Work out the finished part from the listing and answer in its coordinate system (mm). Face numbers are marked on the shaded views. A direction names the side the tool comes from. Round coordinates to 2 decimals unless told otherwise and drop trailing zeros. Loops run counter-clockwise (first coordinate to the right, second up) from the corner with the lowest first, then second, coordinate; pieces in that order, holes last. Notation, with made-up numbers: (48.25, -28.5) - (71.25, -28.5) arc R30 ccw to (71.25, 7.5) - close; hole circle Ø3 at (37.5, 49.5). An arc over 180 degrees is marked (long way). Use CSV: the item, a comma, the result in double quotes. Start each with the question number.
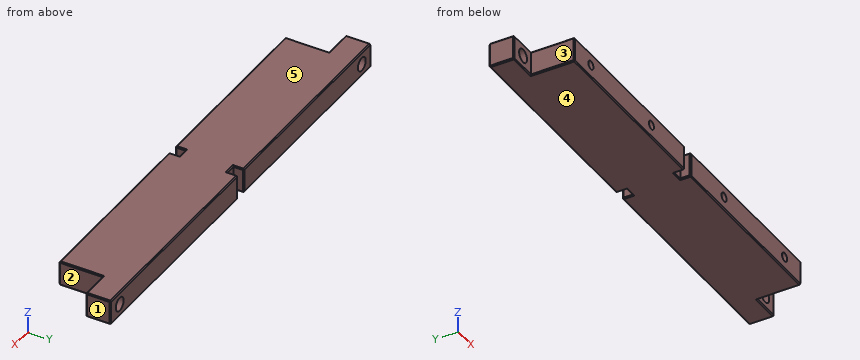
from build123d import *

# Parameters (mm, degrees)
SKETCH_1_W              = 187
SKETCH_1_H              = 33
EXTRUDE_1_DEPTH         = 12
HOLE_WIZARD_M5_1_D      = 4.2
HOLE_WIZARD_M5_1_DEPTH  = 12.4
HOLE_WIZARD_M5_1_TIP    = 1.2618073
SKETCH_8_W              = 5
SKETCH_8_H              = 12
CUT_EXTRUDE_2_DEPTH     = 5
SKETCH_11_W             = 5
SKETCH_11_H             = 5
CUT_EXTRUDE_3_DEPTH     = 96.700052247
SKETCH_12_W             = 14
SKETCH_12_H             = 12
EXTRUDE_2_DEPTH         = 12
HOLE_WIZARD_6_5_6_5_1_D = 6.5
CHAMFER_1_SIZE          = 0.5


with BuildPart() as part:
    # 草图1 → 凸台-拉伸1 (new body)
    with BuildSketch(Plane.XY):
        Rectangle(SKETCH_1_W, SKETCH_1_H)
    extrude(amount=EXTRUDE_1_DEPTH)

    # M5 螺纹孔1
    with Locations(Plane(origin=(0, -16.5, 0), x_dir=(-1, 0, 0), z_dir=(0, -1, 0))):
        with Locations((-80, -6), (-30, -6), (30, -6), (80, -6)):
            Hole(HOLE_WIZARD_M5_1_D / 2, depth=HOLE_WIZARD_M5_1_DEPTH)
            with Locations((0, 0, -(HOLE_WIZARD_M5_1_DEPTH + HOLE_WIZARD_M5_1_TIP / 2))):  # 118° drill point
                Cone(0, HOLE_WIZARD_M5_1_D / 2, HOLE_WIZARD_M5_1_TIP, mode=Mode.SUBTRACT)

    # 草图8 → 切除-拉伸2 (cut)
    with BuildSketch(Plane.XZ.offset(16.5)):
        with Locations((0, 6)):
            Rectangle(SKETCH_8_W, SKETCH_8_H)
    extrude(amount=-CUT_EXTRUDE_2_DEPTH, mode=Mode.SUBTRACT)

    # 草图11 → 切除-拉伸3 (cut, through all)
    with BuildSketch(Plane.XY.offset(12)):
        with Locations((0, 14)):
            Rectangle(SKETCH_11_W, SKETCH_11_H)
    extrude(amount=-CUT_EXTRUDE_3_DEPTH, mode=Mode.SUBTRACT)

    # 草图12 → 凸台-拉伸2 (add)
    with BuildSketch(Plane.XY.offset(12)):
        with Locations((100.5, 10.5)):
            Rectangle(SKETCH_12_W, SKETCH_12_H)
        with Locations((-100.5, 10.5)):
            Rectangle(SKETCH_12_W, SKETCH_12_H)
    extrude(amount=-EXTRUDE_2_DEPTH)

    # Ø6.5 (6.5) 直径孔1 (through all)
    with Locations(Plane(origin=(0, 4.5, 0), x_dir=(-1, 0, 0), z_dir=(0, -1, 0))):
        with Locations((-100, -6), (100, -6)):
            Hole(HOLE_WIZARD_6_5_6_5_1_D / 2)

    # 倒角1
    chamfer_1_edges = [part.edges().sort_by_distance(p)[0] for p in [
        (-48, -16.5, 12),
        (48, -16.5, 0),
        (48, -16.5, 12),
        (-2.5, -14, 0),
        (0, -11.5, 12),
        (-2.5, -14, 12),
        (2.5, -14, 12),
        (0, -11.5, 0),
        (2.5, -14, 0),
        (-2.5, -16.5, 6),
        (2.5, -16.5, 6),
        (93.5, -6, 12),
        (-48, -16.5, 0),
        (-55, 16.5, 0),
        (-55, 16.5, 12),
        (-2.5, 14, 0),
        (55, 16.5, 0),
        (-2.5, 16.5, 6),
        (2.5, 14, 0),
        (2.5, 16.5, 6),
        (0, 11.5, 0),
        (-2.5, 14, 12),
        (0, 11.5, 12),
        (2.5, 14, 12),
        (93.5, -6, 0),
        (100.5, 4.5, 12),
        (107.5, 10.5, 12),
        (100.5, 4.5, 0),
        (107.5, 4.5, 6),
        (107.5, 10.5, 0),
        (107.5, 16.5, 6),
        (93.5, -16.5, 6),
        (-93.5, -16.5, 6),
        (-93.5, -6, 0),
        (-93.5, -6, 12),
        (-107.5, 10.5, 12),
        (-100.5, 4.5, 12),
        (-107.5, 10.5, 0),
        (-107.5, 4.5, 6),
        (-100.5, 4.5, 0),
        (-107.5, 16.5, 6),
        (55, 16.5, 12),
    ]]
    chamfer(chamfer_1_edges, length=CHAMFER_1_SIZE)


solid = part.part
Item 1: A cutting plane is placed at A-A (x = 100). Determine the outline of the cut face in (y, z), plus the area to 3 significant figures.
Item 2: Each of these flat-tipped pins is pushed along its axis until it touches: pin 1 Ø3.5 at (y, z) = (-15, 7.5) entering from +X; pin 2 Ø2 at (y, z) = (-13.5, 8) entering from -X; pin 3 Ø5.5 at (x, z) = (0, 5.5) entering from -Y. Where does it stop, or does it pass through?
Item 3: Find the intervals of material crossed by probe 1 along Z at (x, y) = (-30, -13); probe 2 along X at (y, z) = (15, 3.75); probe 3 along Z at (x, y) = (-100, 7.75), in increasing order. Write a range as [from, to].
Item 4: Which of the six approach directions +Z, -Z, +X, -X, +Y, -Y give full straight-line access (tool end or side, diameter ignored) to the marked faces 1 and 2?
Item 5: The mould has two halves that part along Z. Classify the marked faces 3, 4 and 5: pulls with the +Z half, pulls with the -Z half, needs draft (parallel to the pull), parting line crosses it, or undercut.
Item 6: A cutting plane is placed at B-B (y = 8). Determine the outline of the cut face in (x, z), plus the area to 3 significant figures.
Result sheet:
1,outline,"(4.5, 0.5) - (5, 0) - (16, 0) - (16.5, 0.5) - (16.5, 2.75) - (4.5, 2.75) - close; (4.5, 9.25) - (16.5, 9.25) - (16.5, 11.5) - (16, 12) - (5, 12) - (4.5, 11.5) - close"
1,area,"65.5 mm^2"
2,pin 1,"x = 93.5"
2,pin 2,"x = -93.5"
2,pin 3,"y = -16.25"
3,probe 1,"[0, 3.9], [8.1, 12]"
3,probe 2,"[-107.5, -102.35], [-97.65, -2.5], [2.5, 97.65], [102.35, 107.5]"
3,probe 3,"[0, 2.75], [9.25, 12]"
4,face 1,"+Z, -Z, +X, +Y, -Y"
4,face 2,"+Z, -Z, +X, -Y"
5,face 3,"needs draft"
5,face 4,"pulls with the -Z half"
5,face 5,"pulls with the +Z half"
6,outline,"(-107.5, 0.5) - (-107, 0) - (107, 0) - (107.5, 0.5) - (107.5, 11.5) - (107, 12) - (-107, 12) - (-107.5, 11.5) - close; hole circle Ø6.5 at (-100, 6); hole circle Ø6.5 at (100, 6)"
6,area,"2,510 mm^2"
